Here's how the part is built. I have some questions about the finished solid (model axes, mm). Round coordinates to 2 decimals unless told otherwise and drop trailing zeros. Loops run counter-clockwise (first coordinate to the right, second up) from the corner with the lowest first, then second, coordinate; pieces in that order, holes last. Notation, with made-up numbers: M 38,-38 L 60,-38 A23 ccw 60,0 Z; hole C -32.75,37.5 d6. An arc over 180 degrees is marked long. Answer as a JSON object with one key per item and string values.
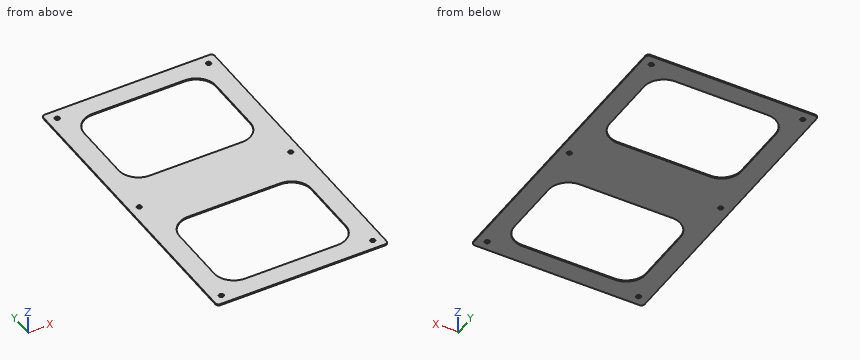
from build123d import *

# Parameters (mm, degrees)
SKETCH_1_W          = 260
SKETCH_1_H          = 460
EXTRUDE_1_DEPTH     = 2
FILLET_1_R          = 5
SKETCH_2_R          = 3.5
CUT_EXTRUDE_1_DEPTH = 529.397577587
CUT_EXTRUDE_2_DEPTH = 529.397577587


with BuildPart() as part:
    # 草图1 → 凸台-拉伸1 (new body)
    with BuildSketch(Plane.XY):
        with Locations((130, -230)):
            Rectangle(SKETCH_1_W, SKETCH_1_H)
    extrude(amount=EXTRUDE_1_DEPTH)

    # 圆角1
    fillet_1_edges = [part.edges().sort_by_distance(p)[0] for p in [
        (0, 0, 1),
        (260, 0, 1),
        (260, -460, 1),
        (0, -460, 1),
    ]]
    fillet(fillet_1_edges, radius=FILLET_1_R)

    # 草图2 → 切除-拉伸1 (cut, through all)
    with BuildSketch(Plane(origin=(0, 0, 0), x_dir=(-1, 0, 0), z_dir=(0, 0, -1))):
        with Locations((-245, -445)):
            Circle(SKETCH_2_R)
        with Locations((-15, -445)):
            Circle(SKETCH_2_R)
        with Locations((-245, -15)):
            Circle(SKETCH_2_R)
        with Locations((-15, -15)):
            Circle(SKETCH_2_R)
        with Locations((-245, -230)):
            Circle(SKETCH_2_R)
        with Locations((-15, -230)):
            Circle(SKETCH_2_R)
    extrude(amount=-CUT_EXTRUDE_1_DEPTH, mode=Mode.SUBTRACT)

    # 草图3 → 切除-拉伸2 (cut, through all)
    with BuildSketch(Plane(origin=(0, 0, 0), x_dir=(-1, 0, 0), z_dir=(0, 0, -1))):
        with BuildLine():
            Line((-60, -430), (-200, -430))
            ThreePointArc((-200, -430), (-221.213203436, -421.213203436), (-230, -400))
            Line((-230, -400), (-230, -310))
            ThreePointArc((-230, -310), (-221.213203436, -288.786796564), (-200, -280))
            Line((-200, -280), (-60, -280))
            ThreePointArc((-60, -280), (-38.786796564, -288.786796564), (-30, -310))
            Line((-30, -310), (-30, -400))
            ThreePointArc((-30, -400), (-38.786796564, -421.213203436), (-60, -430))
        make_face()
        with BuildLine():
            Line((-60, -180), (-200, -180))
            ThreePointArc((-200, -180), (-221.213203436, -171.213203436), (-230, -150))
            Line((-230, -150), (-230, -60))
            ThreePointArc((-230, -60), (-221.213203436, -38.786796564), (-200, -30))
            Line((-200, -30), (-60, -30))
            ThreePointArc((-60, -30), (-38.786796564, -38.786796564), (-30, -60))
            Line((-30, -60), (-30, -150))
            ThreePointArc((-30, -150), (-38.786796564, -171.213203436), (-60, -180))
        make_face()
    extrude(amount=-CUT_EXTRUDE_2_DEPTH, mode=Mode.SUBTRACT)


solid = part.part
Item 1: I want a section at C-C, the plane x = 47. Please give me the cut outline in (y, z).
Resolved:
{"outline": "M -460,0 L -427.04,0 L -427.04,2 L -460,2 Z; M -282.96,0 L -177.04,0 L -177.04,2 L -282.96,2 Z; M -32.96,0 L 0,0 L 0,2 L -32.96,2 Z"}
Item 2: I want a section at A-A, the plane x = 149.5. Please give me the cut outline in (y, z).
Resolved:
{"outline": "M -460,0 L -430,0 L -430,2 L -460,2 Z; M -280,0 L -180,0 L -180,2 L -280,2 Z; M -30,0 L 0,0 L 0,2 L -30,2 Z"}
Item 3: I want a section at B-B, the plane z = 0.65. State how many separate pieces and enclosed holes the cut face has, then the cut area to 3 significant figures.
Resolved:
{"separate pieces": "1", "enclosed holes": "8", "area": "60,900 mm²"}
Item 4: Please list where these lines run through material, in increasing order: probe 1 along X at (y, z) = (-230, 1.25); probe 2 along Y at (x, z) = (15, 0.6); probe 3 along Y at (x, z) = (157.5, 1.5). Write a range as from..to.
Resolved:
{"probe 1": "0..11.5, 18.5..241.5, 248.5..260", "probe 2": "-460..-448.5, -441.5..-233.5, -226.5..-18.5, -11.5..0", "probe 3": "-460..-430, -280..-180, -30..0"}
